Read the model definition and answer for the solid it produces. Units are mm, in the model's axes. A direction names the side the tool comes from. Give positions to 0.01 mm unless a question says otherwise; leave off trailing zeros. Loops run counter-clockwise (first coordinate to the right, second up) from the corner with the lowest first, then second, coordinate; pieces in that order, holes last. Notation, with made-up numbers: (-10, 88.5) - (43, 88.5) arc R14 cw to (43, 111.5) - close; hole circle Ø6 at (37, 55.25). An arc over 180 degrees is marked (long way). Write each question's results on one line, items separated by ' | '. Start each with the question number.
Q1. Find the intervals of material crossed by line 1 (X direction, y = -146, z = 5.75); line 2 (X direction, y = -184.5, z = 18.75); line 3 (Y direction, x = -194.5, z = 9.75), in increasing order. Write a range as from..to.
Q2. The part is cut by section A-A, the plane x = -176. Write down the section's boundary in (y, z).
Q3. The part is cut by section C-C, the plane y = -96. Write down the section's boundary in (x, z).
Q4. For faces 4 (the flat face through (-75, -127, 10)), 5 (the flat face through (-136, -125, 10)), determine the directions among +Z, -Z, +X, -X, +Y, -Y from which every point of the face is accessible in a straight line to the end or side of a thin tool.
Q5. Determine the mould class of faces 1 (the flat face through (-177, -256, 10)), 2 (the cylindrical face through (-176.88, -40.51, 10.14)), 3 (the flat face through (-177, 5, 10)) for opening direction Y: +Y half, -Y half, draft (parallel to the pull), parting line (faces both ways), or undercut.
Q6. The part is cut by section B-B, the plane z = 14.5. Write down the section's boundary in (x, y).
```python
from build123d import *

# Parameters (mm, degrees)
SKETCH_1_W          = 202
SKETCH_1_H          = 261
EXTRUDE_1_DEPTH     = 20
CUT_EXTRUDE_1_DEPTH = 378.710206375


with BuildPart() as part:
    # 草图1 → 凸台-拉伸1 (new body)
    with BuildSketch(Plane.XY):
        with Locations((-176, -125.5)):
            Rectangle(SKETCH_1_W, SKETCH_1_H)
    extrude(amount=EXTRUDE_1_DEPTH)

    # 草图2 → 切除-拉伸1 (cut, through all)
    with BuildSketch(Plane.XY.offset(20)):
        with BuildLine():
            Line((-216, -170.5), (-216, -80.5))
            ThreePointArc((-216, -80.5), (-176, -40.5), (-136, -80.5))
            Line((-136, -80.5), (-136, -170.5))
            ThreePointArc((-136, -170.5), (-176, -210.5), (-216, -170.5))
        make_face()
    extrude(amount=-CUT_EXTRUDE_1_DEPTH, mode=Mode.SUBTRACT)


solid = part.part
```
Check sheet entries:
1) line 1: x = -277..-216, -136..-75 | line 2: x = -277..-213.47, -138.53..-75 | line 3: y = -256..-205.96, -45.04..5
2) outline: (-256, 0) - (-210.5, 0) - (-210.5, 20) - (-256, 20) - close; (-40.5, 0) - (5, 0) - (5, 20) - (-40.5, 20) - close
3) outline: (-277, 0) - (-216, 0) - (-216, 20) - (-277, 20) - close; (-136, 0) - (-75, 0) - (-75, 20) - (-136, 20) - close
4) face 4: +Z, -Z, +X, +Y, -Y | face 5: +Z, -Z
5) face 1: -Y half | face 2: undercut | face 3: +Y half
6) outline: (-277, -256) - (-75, -256) - (-75, 5) - (-277, 5) - close; hole (-216, -170.5) arc R40 ccw to (-136, -170.5) - (-136, -80.5) arc R40 ccw to (-216, -80.5) - close
